Work out the finished part from the listing and answer in its coordinate system (mm). Coordinates: 2 decimals unless noted, no trailing zeros. Order: outer loops, then holes, each group sorted by start corner. A loop starts at its lowest first (then second) coordinate and runs counter-clockwise, first axis right, second up. Notation, with made-up numbers: M 66.25,-25.75 L 122.25,-25.75 A24 ccw 122.25,8.25 Z; hole C 17,65.5 d2. An arc over 180 degrees is marked long. Write item = value, one per line. Start each with the question number.
Q1. Each of these flat-tipped pins is pushed along its axis until it touches: P1, Ø10.5, axis at x = 40, y = -7.5, coming from the +Z side; P2, Ø4.5, axis at y = -24.8, z = 4.75, coming from the -X side; P3, Ø1, axis at y = -22.5, z = 8, coming from the -X side; P4, Ø1, axis at x = 38.5, z = 1, coming from the -Y side. Where does it stop, or does it pass through?
Q2. Find section A-A on x = 10. Give the vertices of the cut face in (y, z).
Q3. Find section D-D on z = 4.25. Give the vertices of the cut face in (x, y), and give its area (3 significant figures).
Q4. Straight lines are drawn through the part: line 1 along X through (y, z) = (-20.75, 4); line 2 along Z through (x, y) = (24, -19.25); line 3 along Y through (x, z) = (18.5, 4.75). For each, find the intervals that lie inside material, in ascending order.
Q5. Find section C-C on x = 58. Give the vertices of the cut face in (y, z).
Q6. Find section B-B on y = -10. Give the vertices of the cut face in (x, z), and give its area (3 significant figures).
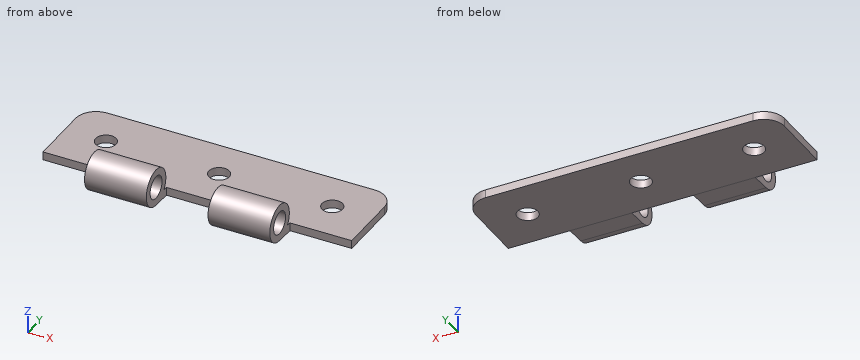
```python
from build123d import *

# Parameters (mm, degrees)
SKETCH1_W           = 75
SKETCH1_H           = 20
SKETCH1_R           = 2.5
BOSS_EXTRUDE1_DEPTH = 2
BOSS_EXTRUDE2_START = -15
BOSS_EXTRUDE2_DEPTH = 15
LPATTERN1_COUNT     = 2
LPATTERN1_PITCH     = 30
FILLET1_R           = 5


with BuildPart() as part:
    # Sketch1 → Boss-Extrude1 (new body)
    with BuildSketch(Plane.XY):
        with Locations((37.5, -10)):
            Rectangle(SKETCH1_W, SKETCH1_H)
        with Locations((10, -10)):
            Circle(SKETCH1_R, mode=Mode.SUBTRACT)
        with Locations((65, -10)):
            Circle(SKETCH1_R, mode=Mode.SUBTRACT)
        with Locations((37.5, -10)):
            Circle(SKETCH1_R, mode=Mode.SUBTRACT)
    extrude(amount=BOSS_EXTRUDE1_DEPTH)

    # Sketch2 → Boss-Extrude2 (add)
    # profile 1 of 2: a face of its own
    with BuildSketch(Plane.ZY.offset(BOSS_EXTRUDE2_START)):
        with BuildLine():
            ThreePointArc((2, -28.361951712), (9.25, -24.8), (2, -21.238048288))
            Line((2, -21.238048288), (2, -24.8))
            Line((2, -24.8), (2, -28.361951712))
        make_face()
        with BuildLine():
            ThreePointArc((7.5, -24.8), (4.75, -27.55), (2, -24.8))
            ThreePointArc((2, -24.8), (4.75, -22.05), (7.5, -24.8))
        make_face(mode=Mode.SUBTRACT)
    # profile 2 of 2: a face of its own
    with BuildSketch(Plane.ZY.offset(BOSS_EXTRUDE2_START)):
        with BuildLine():
            Line((2, -21.238048288), (2, -20))
            Line((2, -20), (0, -20))
            Line((0, -20), (0.255811418, -25.028624118))
            ThreePointArc((0.255811418, -25.028624118), (0.762853744, -26.886304085), (2, -28.361951712))
            Line((2, -28.361951712), (2, -24.8))
            Line((2, -24.8), (2, -21.238048288))
        make_face()
    boss_extrude2 = extrude(amount=-BOSS_EXTRUDE2_DEPTH)

    # LPattern1: Boss-Extrude2 ×2
    with Locations(*[(i * LPATTERN1_PITCH, 0, 0) for i in range(1, LPATTERN1_COUNT)]):
        add(boss_extrude2)

    # Fillet1
    fillet1_edges = [part.edges().sort_by_distance(p)[0] for p in [
        (0, 0, 1),
        (75, 0, 1),
    ]]
    fillet(fillet1_edges, radius=FILLET1_R)


solid = part.part
```
Findings below:
q1.P1 = 2
q1.P2 = through
q1.P3 = 15
q1.P4 = -20
q2.outline = M -20,0 L -12.5,0 L -12.5,2 L -20,2 Z; M -7.5,0 L 0,0 L 0,2 L -7.5,2 Z
q3.outline = M 15,-29.27 L 30,-29.27 L 30,-27.5 L 15,-27.5 Z; M 15,-22.1 L 30,-22.1 L 30,-20.33 L 15,-20.33 Z; M 45,-29.27 L 60,-29.27 L 60,-27.5 L 45,-27.5 Z; M 45,-22.1 L 60,-22.1 L 60,-20.33 L 45,-20.33 Z
q3.area = 106 mm^2
q4.line_1 = 15 to 30, 45 to 60
q4.line_2 = 0 to 2
q4.line_3 = -29.3 to -27.55, -22.05 to -20.3
q5.outline = M -25.03,0.26 L -20,0 L 0,0 L 0,2 L -21.24,2 A4.5 ccw long Z; hole C -24.8,4.75 d5.5
q6.outline = M 0,0 L 7.5,0 L 7.5,2 L 0,2 Z; M 12.5,0 L 35,0 L 35,2 L 12.5,2 Z; M 40,0 L 62.5,0 L 62.5,2 L 40,2 Z; M 67.5,0 L 75,0 L 75,2 L 67.5,2 Z
q6.area = 120 mm^2
